Verification items for the finished model (mm, model axes). A direction names the side the tool comes from. Give positions to 0.01 mm unless a question says otherwise; leave off trailing zeros. Loops run counter-clockwise (first coordinate to the right, second up) from the corner with the lowest first, then second, coordinate; pieces in that order, holes last. Notation, with made-up numbers: M -4,-39 L 33,-39 A26 cw 33,-23 Z; hole C 11,-26 d10. An arc over 180 degrees is marked long. Put each result on its own line as item: value. Start each with the question number.
from build123d import *

# Parameters (mm, degrees)
SKETCH_2_R           = 3
BOSS_EXTRUDE_1_DEPTH = 12
SKETCH_3_R           = 2
BOSS_EXTRUDE_2_DEPTH = 1
BOSS_EXTRUDE_START   = 1.5
SKETCH_4_R           = 2
BOSS_EXTRUDE_3_DEPTH = 1.5
SKETCH_5_R           = 1.25
CUT_EXTRUDE_1_DEPTH  = 6
SKETCH_6_R           = 1.5
CUT_EXTRUDE_2_DEPTH  = 2.5
CUT_EXTRUDE_3_DEPTH  = 6


with BuildPart() as part:
    # Sketch 2 → Boss-Extrude 1 (new body)
    with BuildSketch(Plane(origin=(0, 0, 0), x_dir=(1, 0, 0), z_dir=(0, 1, 0))):
        with Locations(Location((0, 0, 0), (0, 0, 270))):
            Circle(SKETCH_2_R)
    extrude(amount=BOSS_EXTRUDE_1_DEPTH)

    # Sketch 3 → Boss-Extrude 2 (add)
    with BuildSketch(Plane(origin=(0, 12, 0), x_dir=(1, 0, 0), z_dir=(0, 1, 0))):
        with Locations(Location((0, 0, 0), (0, 0, 270))):
            Circle(SKETCH_3_R)
    extrude(amount=BOSS_EXTRUDE_2_DEPTH)

    # Sketch 4 → Boss-Extrude 3 (add)
    with BuildSketch(Plane(origin=(0, 0, 0), x_dir=(-1, 0, 0), z_dir=(0, -1, 0)).offset(BOSS_EXTRUDE_START)):
        with Locations(Location((0, 0, 0), (0, 0, 270))):
            Circle(SKETCH_4_R)
    extrude(amount=-BOSS_EXTRUDE_3_DEPTH)

    # Sketch 5 → Cut-Extrude 1 (cut)
    with BuildSketch(Plane(origin=(0, 13, 0), x_dir=(1, 0, 0), z_dir=(0, 1, 0))):
        with Locations(Location((0, 0, 0), (0, 0, 270))):
            Circle(SKETCH_5_R)
    extrude(amount=-CUT_EXTRUDE_1_DEPTH, mode=Mode.SUBTRACT)

    # Sketch 6 → Cut-Extrude 2 (cut)
    with BuildSketch(Plane(origin=(0, 7, 0), x_dir=(1, 0, 0), z_dir=(0, 1, 0))):
        with Locations(Location((0, 0, 0), (0, 0, 270))):
            Circle(SKETCH_6_R)
    extrude(amount=-CUT_EXTRUDE_2_DEPTH, mode=Mode.SUBTRACT)

    # Sketch 7 → Cut-Extrude 3 (cut)
    with BuildSketch(Plane(origin=(0, -1.5, 0), x_dir=(-1, 0, 0), z_dir=(0, -1, 0))):
        Polygon((-0.97407891, 1.14068851), (-1.385866178, -0.57391196), (0.117566508, -1.495385608), (1.458526276, -0.350287172), (0.783852304, 1.27889623), align=None)
    extrude(amount=-CUT_EXTRUDE_3_DEPTH, mode=Mode.SUBTRACT)


solid = part.part
Q1. Go/stop test with flat-tipped pins: pin 1 (3.5 mm diameter, centred on x = -0.5, z = 0.5, fed in from -Y); pin 2 (1.5 mm diameter, centred on x = 0, z = 0, fed in from -Y). Record where each tip stops, or that it passes through.
Q2. Cross-section at A-A, the plane x = -1. Record the boundary of the cut face in (y, z), then the cut area to 3 significant figures.
Q3. Set-up check for faces 1 (the face through (0.9, 5.92, 2.86)), 2 (the face through (0.64, 1.46, 1.03)), 3 (the face through (-1.22, 10.04, -0.27)): record each of +Z, -Z, +X, -X, +Y, -Y from which the full face is reachable in a straight line by a thin tool's end or side.
Q4. Cross-section at C-C, the plane y = 0.25. Record the boundary of the cut face in (x, z).
Q5. Release check for a two-part mould opening along Y. For faces 4 (the face through (-0.78, 1.46, 0.93)), 5 (the face through (1, 13, 1)), 6 (the face through (0.45, 5.77, 1.43)) record: pulls with the +Y half, pulls with the -Y half, needs draft (parallel to the pull), parting line crosses it, or undercut.
Q6. Cross-section at D-D, the plane y = 6.75. Record the boundary of the cut face in (x, z), then the cut area to 3 significant figures.
Q7. Scan lines: L1, parallel to X at y = 5.2, z = 0; L2, parallel to Y at x = 2.6, z = 1.2; L3, parallel to X at y = 11.35, z = 0. Record each from-to range of solid material in increasing order.
Q8. Cross-section at B-B, the plane z = 0.05. Record the boundary of the cut face in (x, y), then the cut area to 3 significant figures.
Ans:
1. pin 1: stops at y = -1.5
1. pin 2: passes through
2. outline: M -1.5,-1.73 L 0,-1.73 L 0,-2.83 L 12,-2.83 L 12,-1.73 L 13,-1.73 L 13,-0.75 L 7,-0.75 L 7,-1.12 L 4.5,-1.12 L 4.5,-0.76 L -1.5,-0.76 Z; M -1.5,0.74 L 4.5,0.74 L 4.5,1.12 L 7,1.12 L 7,0.75 L 13,0.75 L 13,1.73 L 12,1.73 L 12,2.83 L 0,2.83 L 0,1.73 L -1.5,1.73 Z
2. area: 53.0 mm^2
3. face 1: +Y, -Y
3. face 2: -Y
3. face 3: +Y
4. outline: C 0,0 d6; hole M -1.46,0.35 L -0.78,-1.28 L 0.97,-1.14 L 1.39,0.57 L -0.12,1.5 Z
5. face 4: needs draft
5. face 5: pulls with the +Y half
5. face 6: undercut
6. outline: C 0,0 d6; hole C 0,0 d3
6. area: 21.2 mm^2
7. L1: x = -3 to -1.5, 1.5 to 3
7. L2: y = 0 to 12
7. L3: x = -3 to -1.25, 1.25 to 3
8. outline: M -3,0 L -2,0 L -2,-1.5 L -1.33,-1.5 L -1.33,4.5 L -1.5,4.5 L -1.5,7 L -1.25,7 L -1.25,13 L -2,13 L -2,12 L -3,12 Z; M 1.25,7 L 1.5,7 L 1.5,4.5 L 1.26,4.5 L 1.26,-1.5 L 2,-1.5 L 2,0 L 3,0 L 3,12 L 2,12 L 2,13 L 1.25,13 Z
8. area: 43.9 mm^2
